Geometry check sheet. Reference: drawing and pictorial views, mm from the part's lowest x, y, z. A direction names the side the tool comes from. Give positions to 0.01 mm unless a question says otherwise; leave off trailing zeros. Write each loop counter-clockwise with the first axis right and the second up, starting at its lowest first coordinate (ties: lowest second). Pieces come first, ordered by that corner, then holes. Notation, with made-up numbers: M -13.5,4.25 L 24.5,4.25 A38 cw 24.5,43.25 Z; hole C 56.25,47.5 d9. An arc over 180 degrees is marked long. Write each question's results on one line, items separated by ' | '. Start each with the question number.
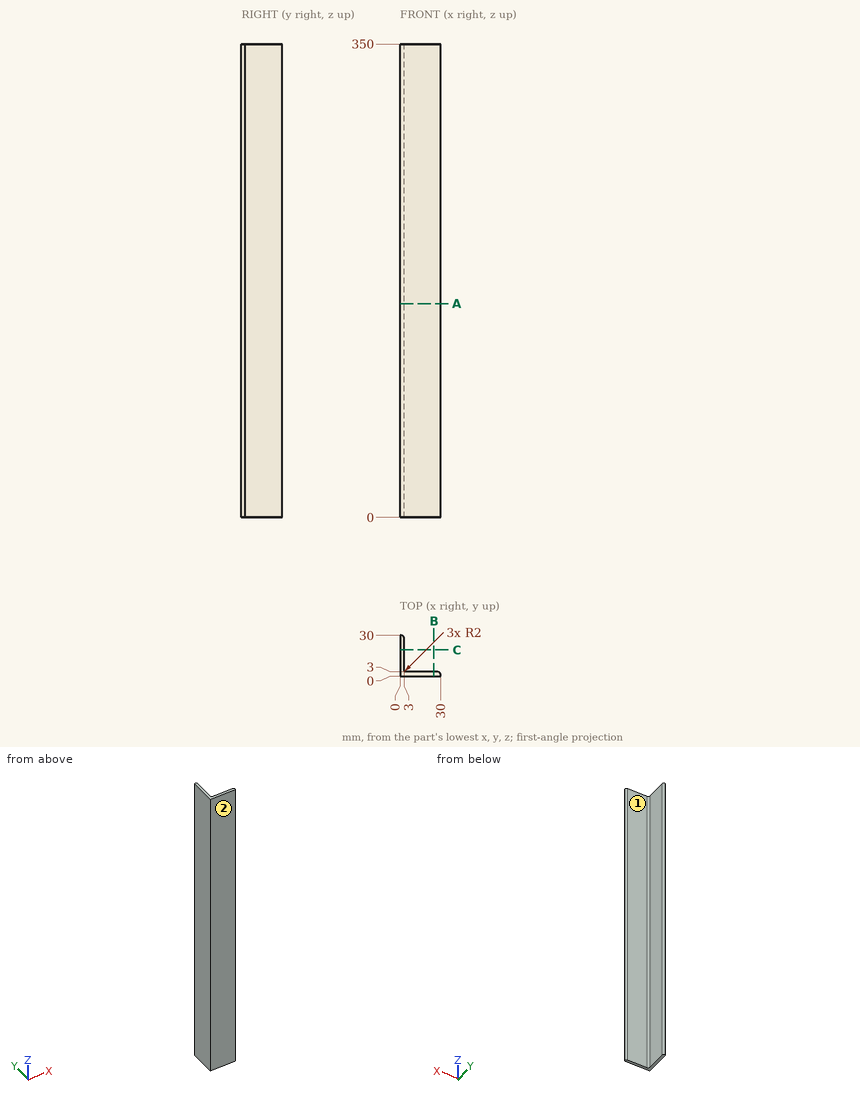
Q1. Section check B-B on x = 25. Record the boundary of the cut face in (y, z).
Q2. Depth check by flat-ended pin: pin 1 Ø8 at (x, z) = (15, 280) entering from +Y; pin 2 Ø2 at (y, z) = (8, 36) entering from +X. Enter the tip coordinate at first touch or a pass-through.
Q3. Section check A-A on z = 158. Record the boundary of the cut face in (x, y).
Q4. Scan lines: L1, parallel to X at y = 5.25, z = 122; L2, parallel to Y at x = 3.25, z = 128.5. Record each from-to range of solid material in increasing order.
Q5. Tool access check on the marked faces 1 and 2. Record the directions out of +Z, -Z, +X, -X, +Y, -Y that give a thin tool (end or side, any length) a straight path to the whole face; none if there is none.
Check result:
1) outline: M 0,0 L 3,0 L 3,350 L 0,350 Z
2) pin 1: y = 3 | pin 2: x = 3
3) outline: M 0,0 L 30,0 L 30,1 A2 ccw 28,3 L 5,3 A2 cw 3,5 L 3,28 A2 ccw 1,30 L 0,30 Z
4) L1: 0 to 3 | L2: 0 to 4.03
5) face 1: +Z, -Z, +X, +Y | face 2: +Z, -Z, +X, -X, -Y
